Can you work these out from the model? Positions are in its coordinate system, mm. Face numbers are marked on the shaded views. A direction names the side the tool comes from. Give positions to 0.01 mm unless a question says otherwise; leave off trailing zeros. Loops run counter-clockwise (first coordinate to the right, second up) from the corner with the lowest first, then second, coordinate; pieces in that order, holes last. Notation, with made-up numbers: M 13.5,-22 L 44.5,-22 A20 cw 44.5,9 Z; hole C -20.5,-16 d2. An arc over 180 degrees is marked long. Put each result on its own line as item: value. Start each with the question number.
1) Imagine slicing it at A-A (x = 66). Write out the boundary of the cut face in (y, z), then the cut area to 3 significant figures.
2) Please list where these lines run through material, in increasing order: line 1 along Z through (x, y) = (46, 189); line 2 along Z through (x, y) = (41, 108); line 3 along Y through (x, z) = (80, -50). Write a range as from..to.
3) For the marked faces 5 and 6, which set-ups out of +Z, -Z, +X, -X, +Y, -Y let a thin tool reach every point of the face, with its end or its side?
4) For P1, Ø4, axis at x = 37, y = 93, coming from the -Z side, with a flat end and sliding along its axis, tell me the tip position at first contact or that it passes through.
5) Imagine slicing it at D-D (x = 9). Write out the boundary of the cut face in (y, z), then the cut area to 3 significant figures.
6) Imagine slicing it at C-C (z = -35). Write out the boundary of the cut face in (x, y), then the cut area to 3 significant figures.
7) If we mould it in two halves opening along Y, with no side actions, what happens to the marked faces 1, 2, 3 and 4? For each: +Y half, -Y half, draft (parallel to the pull), parting line (faces both ways), or undercut.
8) Imagine slicing it at B-B (z = -47). Write out the boundary of the cut face in (x, y), then the cut area to 3 significant figures.
from build123d import *

# Parameters (mm, degrees)
C_20A_1_DEPTH       = 100
CUT_EXTRUDE_1_DEPTH = 16


with BuildPart() as part:
    # Sketch1 → C 槽 20A(1) (new body)
    with BuildSketch(Plane(origin=(0, 0, 0), x_dir=(0, 0, -1), z_dir=(1, 0, 0))):
        with BuildLine():
            Line((73, 200), (0, 200))
            Line((0, 200), (0, 0))
            Line((0, 0), (73, 0))
            Line((73, 0), (73, 2.579337993))
            ThreePointArc((73, 2.579337993), (71.58729654, 6.259556328), (68.074906548, 8.049208417))
            Line((68.074906548, 8.049208417), (16.850186904, 13.433143402))
            ThreePointArc((16.850186904, 13.433143402), (9.82540692, 17.012447581), (7, 24.372884251))
            Line((7, 24.372884251), (7, 175.627115749))
            ThreePointArc((7, 175.627115749), (9.82540692, 182.987552419), (16.850186904, 186.566856598))
            Line((16.850186904, 186.566856598), (68.074906548, 191.950791583))
            ThreePointArc((68.074906548, 191.950791583), (71.58729654, 193.740443672), (73, 197.420662007))
            Line((73, 197.420662007), (73, 200))
        make_face()
    extrude(amount=C_20A_1_DEPTH)

    # 草图2 → 切除-拉伸1 (cut)
    with BuildSketch(Plane(origin=(0, 200, 0), x_dir=(1, 0, 0), z_dir=(0, 1, 0))):
        with BuildLine():
            Line((20, 44), (80, 44))
            ThreePointArc((80, 44), (89, 35), (80, 26))
            Line((80, 26), (20, 26))
            ThreePointArc((20, 26), (11, 35), (20, 44))
        make_face()
    extrude(amount=-CUT_EXTRUDE_1_DEPTH, mode=Mode.SUBTRACT)


solid = part.part
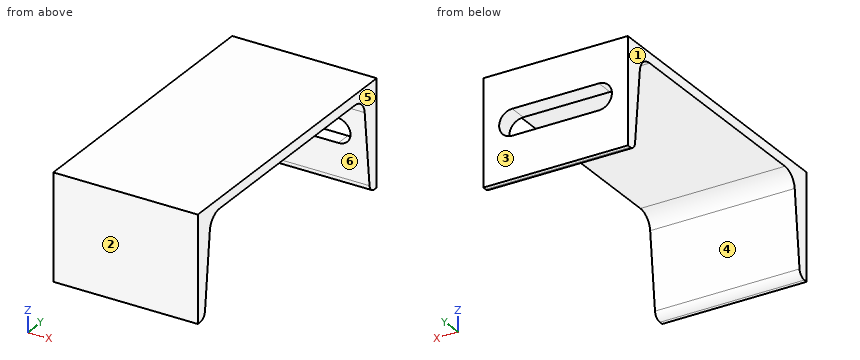
Recorded:
1. outline: M 0,-73 L 2.58,-73 A5.5 ccw 8.05,-68.07 L 13.43,-16.85 A11 cw 24.37,-7 L 175.63,-7 A11 cw 186.57,-16.85 L 187.53,-26 L 200,-26 L 200,0 L 0,0 Z; M 189.42,-44 L 191.95,-68.07 A5.5 ccw 197.42,-73 L 200,-73 L 200,-44 Z
1. area: 2,670 mm²
2. line 1: -26..0
2. line 2: -7..0
2. line 3: 0..9.95, 190.05..200
3. face 5: +Z, -Z, +X, +Y, -Y
3. face 6: -Z, +X, -X
4. P1: z = -7
5. outline: M 0,-73 L 2.58,-73 A5.5 ccw 8.05,-68.07 L 13.43,-16.85 A11 cw 24.37,-7 L 175.63,-7 A11 cw 186.57,-16.85 L 191.95,-68.07 A5.5 ccw 197.42,-73 L 200,-73 L 200,0 L 0,0 Z
5. area: 2,880 mm²
6. outline: M 0,0 L 100,0 L 100,11.53 L 0,11.53 Z; M 0,188.47 L 11,188.47 L 11,200 L 0,200 Z; M 89,188.47 L 100,188.47 L 100,200 L 89,200 Z
6. area: 1,410 mm²
7. face 1: draft
7. face 2: -Y half
7. face 3: +Y half
7. face 4: undercut
8. outline: M 0,0 L 100,0 L 100,10.26 L 0,10.26 Z; M 0,189.74 L 100,189.74 L 100,200 L 0,200 Z
8. area: 2,050 mm²
